Can you work these out from the model? Positions are in its coordinate system, mm. Give positions to 0.01 mm unless a question says otherwise; leave off trailing zeros. Write each loop counter-clockwise with the first axis right and the second up, starting at its lowest first coordinate (ties: lowest second). Pieces come first, ordered by that corner, then holes.
```python
from build123d import *

# Parameters (mm, degrees)
SKETCH1_W           = 53.848
SKETCH1_H           = 50.8
SKETCH1_R           = 7.1374
BOSS_EXTRUDE1_DEPTH = 4


with BuildPart() as part:
    # Sketch1 → Boss-Extrude1 (new, symmetric)
    with BuildSketch(Plane.XY):
        with Locations((-11.176, 0)):
            Rectangle(SKETCH1_W, SKETCH1_H)
        Circle(SKETCH1_R, mode=Mode.SUBTRACT)
    extrude(amount=BOSS_EXTRUDE1_DEPTH, both=True)


solid = part.part
```
1) If we mould it in two halves opening along Y, with no side actions, what happens to faces 1 (the face through (-7.13, 0.31, -0.06)), 2 (the face through (15.748, 0, 0)), 3 (the face through (-12, 25.4, 0))? For each: +Y half, -Y half, draft (parallel to the pull), parting line (faces both ways), or undercut.
Values follow:
face 1: undercut
face 2: draft
face 3: +Y half
2) Please list where these lines run through material, in increasing order: L1, parallel to Y at x = 0, z = -0.75; L2, parallel to X at y = 3, z = -0.5; L3, parallel to Y at x = -2.5, z = 1.75.
Values follow:
L1: y = -25.4 to -7.14, 7.14 to 25.4
L2: x = -38.1 to -6.48, 6.48 to 15.75
L3: y = -25.4 to -6.69, 6.69 to 25.4
3) Suppose I cut it at B-B on x = 0. Write out the boundary of the cut face in (y, z).
Values follow:
outline: (-25.4, -4) - (-7.14, -4) - (-7.14, 4) - (-25.4, 4) - close; (7.14, -4) - (25.4, -4) - (25.4, 4) - (7.14, 4) - close
4) Suppose I cut it at A-A on y = 0. Write out the boundary of the cut face in (x, z).
Values follow:
outline: (-38.1, -4) - (-7.14, -4) - (-7.14, 4) - (-38.1, 4) - close; (7.14, -4) - (15.75, -4) - (15.75, 4) - (7.14, 4) - close
5) Suppose I cut it at C-C on z = -1.25. Write out the boundary of the cut face in (x, y).
Values follow:
outline: (-38.1, -25.4) - (15.75, -25.4) - (15.75, 25.4) - (-38.1, 25.4) - close; hole circle Ø14.27 at (0, 0)
